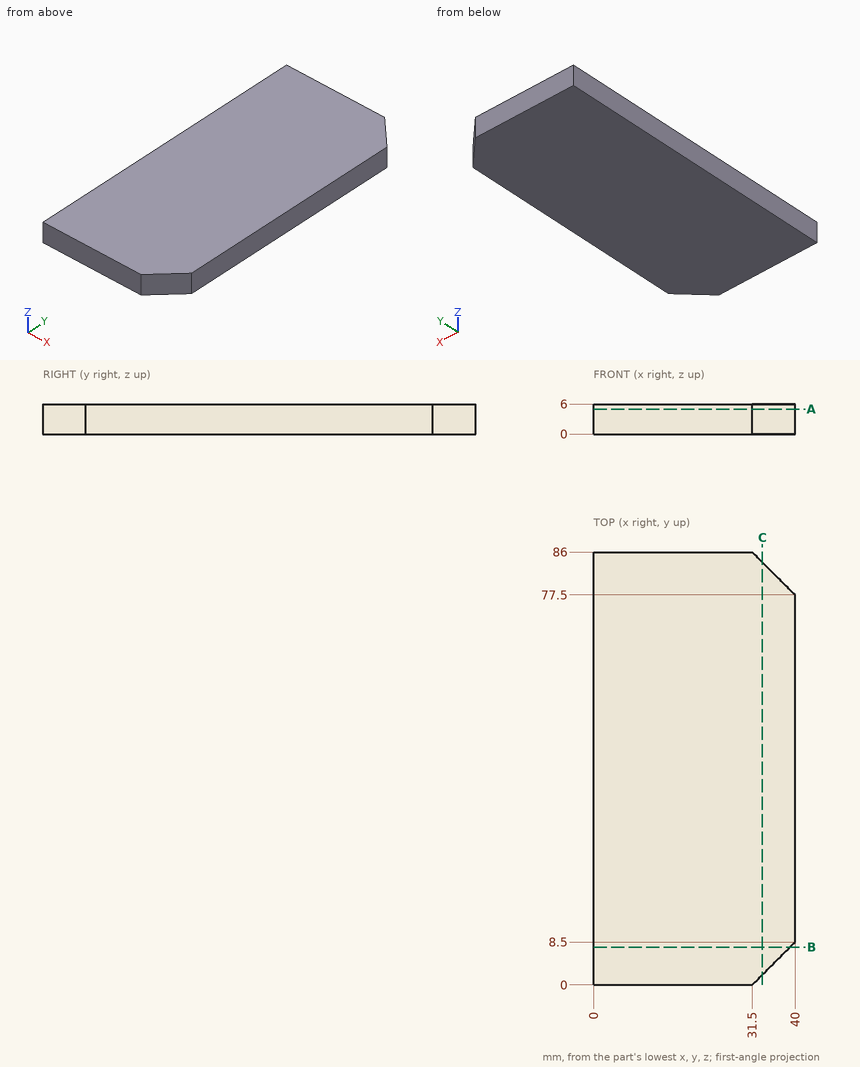
The drawing under review shows one solid part. Ordinate dimensions are in mm from its lowest x, y, z. Round coordinates to 2 decimals unless told otherwise and drop trailing zeros. Order: outer loops, then holes, each group sorted by start corner. A loop starts at its lowest first (then second) coordinate and runs counter-clockwise, first axis right, second up. Notation, with made-up numbers: (65.25, -4) - (120.25, -4) arc R12 ccw to (120.25, 12) - close; hole circle Ø7 at (33, -6). An arc over 180 degrees is marked (long way). Return JSON: item names as keys, results as strings.
Q1. Consider section C-C on x = 33.5. Write out the cut boundary in (y, z).
Computed values:
{"outline": "(2, 0) - (84, 0) - (84, 6) - (2, 6) - close"}
Q2. Wall thickness on L1, parallel to X at y = 80, z = 0.5; L2, parallel to X at y = 81, z = 3.25; L3, parallel to Y at x = 34, z = 2: over which ranges is each line inside the solid? List them lowest first. Write a range as [from, to].
Computed values:
{"L1": "x = [0, 37.5]", "L2": "x = [0, 36.5]", "L3": "y = [2.5, 83.5]"}
Q3. For pin 1 Ø1.5 at (x, z) = (34.5, 1) entering from +Y, flat-tipped, find the tip position at first contact; note if it passes through.
Computed values:
{"pin 1": "stops at y = 83.75"}
Q4. Consider section A-A on z = 5. Write out the cut boundary in (x, y), plus the area to 3 significant figures.
Computed values:
{"outline": "(0, 0) - (31.5, 0) - (40, 8.5) - (40, 77.5) - (31.5, 86) - (0, 86) - close", "area": "3,370 mm2"}
Q5. Consider section B-B on y = 7.5. Write out the cut boundary in (x, z), plus the area to 3 significant figures.
Computed values:
{"outline": "(0, 0) - (39, 0) - (39, 6) - (0, 6) - close", "area": "234 mm2"}
